Part model, mm, in its own coordinate system. A direction names the side the tool comes from. Round coordinates to 2 decimals unless told otherwise and drop trailing zeros. Write each loop counter-clockwise with the first axis right and the second up, starting at its lowest first coordinate (ties: lowest second). Pieces come first, ordered by that corner, then holes. Notation, with made-up numbers: (19.25, 27) -> (43.25, 27) arc R16 cw to (43.25, 43) -> close; hole circle Ø11 at (10.25, -13.75). An arc over 180 degrees is marked (long way). Use CSV: the item, a comma, the result in double quotes. Start each with the question number.
```python
from build123d import *

# Parameters (mm, degrees)
FLANGE_PROFILE_90X_30_R     = 45
FLANGE_PROFILE_90X_30_R_2   = 15
FLANGE_90_DEPTH             = 14.2
MOUNTING_HOLES_SKETCH_R     = 6.25
FLANGE_MOUNTING_HOLES_DEPTH = 66.204601065
FLANGE_EDGE_FILLET_R2_R     = 2
HUB_PROFILE_40X_30_R        = 20
HUB_PROFILE_40X_30_R_2      = 15
HUB_40_DEPTH                = 44.2
COLLAR_PROFILE_50X_30_R     = 25
COLLAR_PROFILE_50X_30_R_2   = 15
COLLAR_50_DEPTH             = 6
SOCKET_PROFILE_50X_38_R     = 25
SOCKET_PROFILE_50X_38_R_2   = 19
SOCKET_50_DEPTH             = 24
FLANGE_CHAMFER_SIZE         = 3
FLANGE_CHAMFER_SIZE2        = 3.5
HUB_ROOT_FILLET_R2_R        = 2
SOCKET_EDGE_FILLET_R2_5_R   = 2.5


with BuildPart() as part:
    # Flange Profile Ø90xØ30 → Flange Ø90 (new body)
    with BuildSketch(Plane.XY):
        Circle(FLANGE_PROFILE_90X_30_R)
        Circle(FLANGE_PROFILE_90X_30_R_2, mode=Mode.SUBTRACT)
    extrude(amount=FLANGE_90_DEPTH)

    # Mounting Holes Sketch → Flange Mounting Holes (cut, through all)
    with BuildSketch(Plane.XY.offset(14.2)):
        with Locations((0, 32.5)):
            Circle(MOUNTING_HOLES_SKETCH_R)
        with Locations((-32.5, 0)):
            Circle(MOUNTING_HOLES_SKETCH_R)
        with Locations(Location((32.5, 0, 0), (0, 0, 180))):
            Circle(MOUNTING_HOLES_SKETCH_R)
        with Locations(Location((0, -32.5, 0), (0, 0, 180))):
            Circle(MOUNTING_HOLES_SKETCH_R)
    extrude(amount=-FLANGE_MOUNTING_HOLES_DEPTH, mode=Mode.SUBTRACT)

    # Flange Edge Fillet R2
    flange_edge_fillet_r2_edges = [part.edges().sort_by_distance(p)[0] for p in [
        (-45, 0, 14.2),
    ]]
    fillet(flange_edge_fillet_r2_edges, radius=FLANGE_EDGE_FILLET_R2_R)

    # Hub Profile Ø40xØ30 → Hub Ø40 (add)
    with BuildSketch(Plane.XY.offset(14.2)):
        Circle(HUB_PROFILE_40X_30_R)
        Circle(HUB_PROFILE_40X_30_R_2, mode=Mode.SUBTRACT)
    extrude(amount=HUB_40_DEPTH)

    # Collar Profile Ø50xØ30 → Collar Ø50 (add)
    with BuildSketch(Plane.XY.offset(58.4)):
        Circle(COLLAR_PROFILE_50X_30_R)
        Circle(COLLAR_PROFILE_50X_30_R_2, mode=Mode.SUBTRACT)
    extrude(amount=COLLAR_50_DEPTH)

    # Socket Profile Ø50xØ38 → Socket Ø50 (add)
    with BuildSketch(Plane.XY.offset(64.4)):
        Circle(SOCKET_PROFILE_50X_38_R)
        Circle(SOCKET_PROFILE_50X_38_R_2, mode=Mode.SUBTRACT)
    extrude(amount=SOCKET_50_DEPTH)

    # Flange Chamfer
    flange_chamfer_edges = [part.edges().sort_by_distance(p)[0] for p in [
        (-15, 0, 0),
    ]]
    flange_chamfer_side = [part.faces().sort_by_distance(p)[0] for p in [
        (-15, 0, 32.2),
    ]]
    chamfer(flange_chamfer_edges, length=FLANGE_CHAMFER_SIZE, length2=FLANGE_CHAMFER_SIZE2, reference=flange_chamfer_side[0])

    # Hub Root Fillet R2
    hub_root_fillet_r2_edges = [part.edges().sort_by_distance(p)[0] for p in [
        (-20, 0, 14.2),
    ]]
    fillet(hub_root_fillet_r2_edges, radius=HUB_ROOT_FILLET_R2_R)

    # Socket Edge Fillet R2.5
    socket_edge_fillet_r2_5_edges = [part.edges().sort_by_distance(p)[0] for p in [
        (-25, 0, 88.4),
        (-19, 0, 88.4),
    ]]
    fillet(socket_edge_fillet_r2_5_edges, radius=SOCKET_EDGE_FILLET_R2_5_R)


solid = part.part
```
1. Pull direction Y, two halves, no side cores. Call faces 4 (the flat face through (-20, 10, 14.2)), 5 (the cylindrical face through (20.765, -39.923, 6.015)), 6 (the cylindrical face through (-38.744, 0.275, 7.199)): released by +Y, released by -Y, zero draft, split by the parting line, or undercut.
2. Flat gauge pins, fed straight in: pin 1 (4 mm diameter, centred on y = -33.5, z = 12, fed in from +X); pin 2 (14.5 mm diameter, centred on x = 0, y = 32.5, fed in from +Z); pin 3 (8 mm diameter, centred on y = -21, z = 41, fed in from -X). Where does each tip first touch, or does it go through?
3. Band-saw the part on C-C (z = 82.5). List the corners of the cut face in (x, y).
4. Which spindle directions (+Z, -Z, +X, -X, +Y, -Y) get a long thin tool onto all of the face, cutting with end or side? Do faces 1 (the cylindrical face through (38.744, -0.275, 7.199)), 2 (the cylindrical face through (23.846, 7.509, 71.958)), 3 (the cylindrical face through (-4.336, -19.524, 37.005)). Say none if no direction does.
5. Band-saw the part on A-A (z = 6.5). List the corners of the cut face in (x, y), then the cut area to 3 significant figures.
6. Drill centre lines: line 1 along Y through (x, z) = (0, 80); line 2 along Z through (x, y) = (-20, 36); line 3 along Y through (x, z) = (-11, 31). Where is each one in solid material? Low to high. Write a range as [from, to].
7. Band-saw the part on B-B (y = 0). Give the number of separate pieces and of enclosed holes in the cut face, then the cut area to 3 significant figures.
Answers below:
1,face 4,"zero draft"
1,face 5,"split by the parting line"
1,face 6,"undercut"
2,pin 1,"stops at x = 32.14"
2,pin 2,"stops at z = 14.2"
2,pin 3,"stops at x = -10.54"
3,outline,"circle Ø50 at (0, 0); hole circle Ø38 at (0, 0)"
4,face 1,"+Z, -Z"
4,face 2,"+Z"
4,face 3,"none"
5,outline,"circle Ø90 at (0, 0); hole circle Ø12.5 at (-32.5, 0); hole circle Ø30 at (0, 0); hole circle Ø12.5 at (0, -32.5); hole circle Ø12.5 at (0, 32.5); hole circle Ø12.5 at (32.5, 0)"
5,area,"5,160 mm^2"
6,line 1,"y = [-25, -19], [19, 25]"
6,line 2,"z = [0, 14.2]"
6,line 3,"y = [-16.7, -10.2], [10.2, 16.7]"
7,separate pieces,"4"
7,enclosed holes,"0"
7,area,"1,330 mm^2"
